```python
from build123d import *

# Parameters (mm, degrees)
EXTRUDE_1_DEPTH     = 60
EXTRUDE_2_DEPTH     = 60
SKETCH_3_R          = 10
CUT_EXTRUDE_1_DEPTH = 60


with BuildPart() as part:
    # 草图1 → 凸台-拉伸1 (new body)
    with BuildSketch(Plane.XY):
        Polygon((0, 0), (0, 60), (-10, 60), (-10, -10), (60, -10), (60, 0), align=None)
    extrude(amount=EXTRUDE_1_DEPTH)

    # 草图2 → 凸台-拉伸2 (add)
    with BuildSketch(Plane.XY):
        Polygon((0, 60), (-40.710678119, 100.710678119), (-47.781745931, 93.639610307), (-10, 55.857864376), (-10, 60), align=None)
        Polygon((60, 0), (100.710678119, -40.710678119), (93.639610307, -47.781745931), (55.857864376, -10), (60, -10), align=None)
    extrude(amount=EXTRUDE_2_DEPTH)

    # 草图3 → 切除-拉伸1 (cut)
    with BuildSketch(Plane(origin=(22.928932188, 22.928932188, 0), x_dir=(0, 0, 1), z_dir=(-0.7071067811865501, -0.7071067811865449, 0))):
        with Locations(Location((30, 75, 0), (0, 0, 270))):
            Circle(SKETCH_3_R)
        with Locations(Location((30, -75, 0), (0, 0, 270))):
            Circle(SKETCH_3_R)
    extrude(amount=-CUT_EXTRUDE_1_DEPTH, mode=Mode.SUBTRACT)


solid = part.part
```
CAD build for the part. Positions are in the model's coordinates, mm. A direction names the side the tool comes from. Give positions to 0.01 mm unless a question says otherwise; leave off trailing zeros. Write each loop counter-clockwise with the first axis right and the second up, starting at its lowest first coordinate (ties: lowest second). Pieces come first, ordered by that corner, then holes. Notation, with made-up numbers: M 53,37.25 L 95,37.25 A30 cw 95,59.25 Z; hole C -3.75,-5.5 d3. An arc over 180 degrees is marked long. Return JSON: item names as keys, results as strings. Group by question number.
(1) Drill centre lines: L1, parallel to X at y = 33, z = 9.5; L2, parallel to Y at x = -22.5, z = 12.5. Where is each one in solid material? Low to high. Write a range as [from, to].
(2) Band-saw the part on B-B (z = 56). Give the cut face in (x, y).
(3) Mould opens along Z. For faces 4 (the face through (-1, 21, 0)), 5 (the face through (-28.151, 80.981, 20.238)), 6 (the face through (0, 30, 30)) say: pulls with the +Z half, pulls with the -Z half, needs draft (parallel to the pull), parting line crosses it, or undercut.
(4) Band-saw the part on A-A (z = 22). Give the cut face in (x, y).
(5) Flat gauge pins, fed straight in: pin 1 Ø8 at (x, z) = (-6, 36) entering from +Y; pin 2 Ø18 at (x, z) = (14.5, 27) entering from -Y; pin 3 Ø4 at (y, z) = (29, 34) entering from -X; pin 4 Ø1.5 at (x, y) = (-11.5, 37) entering from -Z. Where does each tip first touch, or does it go through?
(6) Band-saw the part on C-C (x = 34.5). Give the cut face in (y, z), and give its area (3 significant figures).
(7) 3-axis set-ups, long thin cutter, end or side, ignore diameter. For faces 1 (the face through (-44.2, 97.22, 29.58)), 2 (the face through (30, 0, 30)), 3 (the face through (22, -10, 30)): which of +Z, -Z, +X, -X, +Y, -Y reach the whole face in a straight line?
Entries:
{
 "1": {"L1": "x = [-10, 0]", "L2": "y = [68.36, 82.5]"},
 "2": {"outline": "M -47.78,93.64 L -10,55.86 L -10,-10 L 55.86,-10 L 93.64,-47.78 L 100.71,-40.71 L 60,0 L 0,0 L 0,60 L -40.71,100.71 Z"},
 "3": {"face 4": "pulls with the -Z half", "face 5": "undercut", "face 6": "needs draft"},
 "4": {"outline": "M -47.78,93.64 L -34.35,80.2 L -27.28,87.28 L -40.71,100.71 Z; M -25.86,71.72 L -10,55.86 L -10,-10 L 55.86,-10 L 71.72,-25.86 L 78.79,-18.79 L 60,0 L 0,0 L 0,60 L -18.79,78.79 Z; M 80.2,-34.35 L 93.64,-47.78 L 100.71,-40.71 L 87.28,-27.28 Z"},
 "5": {"pin 1": "stops at y = 70", "pin 2": "stops at y = -10", "pin 3": "stops at x = -10", "pin 4": "passes through"},
 "6": {"outline": "M -10,0 L 0,0 L 0,60 L -10,60 Z", "area": "600 mm^2"},
 "7": {"face 1": "+Z, -Z, -X, +Y", "face 2": "+Z, -Z, +X, +Y", "face 3": "+Z, -Z, -X, -Y"}
}
